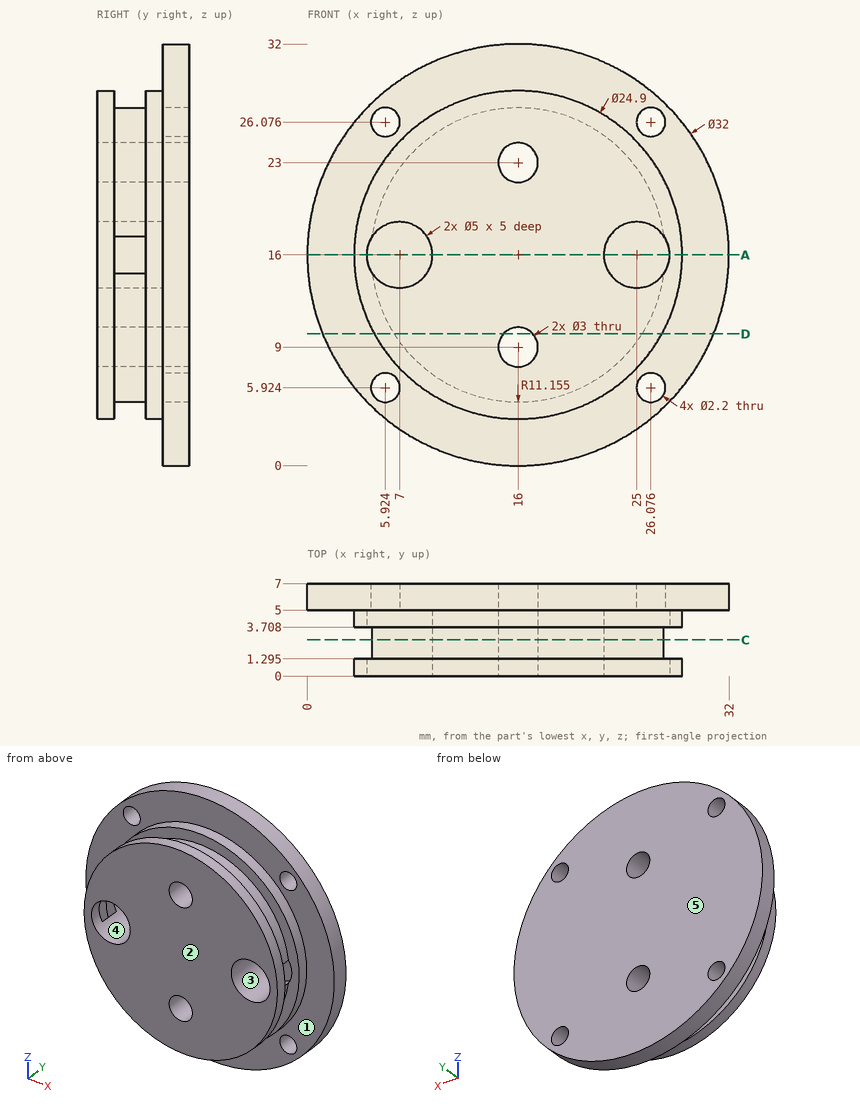
Check sheet for the drawn part. Datum: minimum x, y, z corner. Units: mm. A direction names the side the tool comes from. Give positions to 0.01 mm unless a question says otherwise; leave off trailing zeros. Order: outer loops, then holes, each group sorted by start corner. A loop starts at its lowest first (then second) coordinate and runs counter-clockwise, first axis right, second up. Notation, with made-up numbers: (47, 17) - (81, 17) arc R29 ccw to (81, 48) - close; hole circle Ø7 at (-14, -11.5). An arc over 180 degrees is marked (long way). Answer as a JSON object with one key per item and string values.
(1) Depth check by flat-ended pin: pin 1 Ø2.5 at (x, z) = (8, 17) entering from -Y; pin 2 Ø1 at (y, z) = (1, 26.5) entering from +X (1 decimal); pin 3 Ø3.5 at (x, z) = (5.92, 5.92) entering from -Y; pin 4 Ø4 at (x, y) = (13.5, 5) entering from -Z. Enter the tip coordinate at first touch or a pass-through.
Report:
{"pin 1": "y = 0", "pin 2": "x = 23.4", "pin 3": "y = 5", "pin 4": "z = 0.01"}
(2) Cross-section at A-A (z = 16). State how many separate pieces and enclosed holes the cut face has, then the cut area to 3 significant figures.
Report:
{"separate pieces": "3", "enclosed holes": "0", "area": "134 mm^2"}
(3) Cross-section at D-D (z = 10). Record the cut outline in (x, y) (1 decimal).
Report:
{"outline": "(1.2, 5) - (5.1, 5) - (5.1, 3.7) - (6.6, 3.7) - (6.6, 1.3) - (5.1, 1.3) - (5.1, 0) - (14.9, 0) - (14.9, 7) - (1.2, 7) - close; (17.1, 0) - (26.9, 0) - (26.9, 1.3) - (25.4, 1.3) - (25.4, 3.7) - (26.9, 3.7) - (26.9, 5) - (30.8, 5) - (30.8, 7) - (17.1, 7) - close"}
(4) Material ranges on line 1 (X direction, y = 0.5, z = 16); line 2 (X direction, y = 4.5, z = 14); line 3 (Z direction, x = 5.5, y = 5.5), recorded low to high.
Report:
{"line 1": "3.55 to 4.5, 9.5 to 22.5, 27.5 to 28.45", "line 2": "3.71 to 5.5, 8.5 to 23.5, 26.5 to 28.29", "line 3": "3.93 to 4.91, 6.94 to 25.06, 27.09 to 28.07"}
(5) Draft check along X on the marked faces 3, 4 and 5. Enter one of: released by +X, released by -X, zero draft, split by the parting line, or undercut.
Report:
{"face 3": "undercut", "face 4": "undercut", "face 5": "zero draft"}
(6) Tool access check on the marked faces 1 and 2. Record the directions out of +Z, -Z, +X, -X, +Y, -Y that give a thin tool (end or side, any length) a straight path to the whole face; none if there is none.
Report:
{"face 1": "-Y", "face 2": "+Z, -Z, +X, -X, -Y"}
(7) Cross-section at C-C (y = 2.75). Record the cut outline in (x, z) (1 decimal).
Report:
{"outline": "(4.9, 14.6) arc R11.2 ccw to (27.1, 14.6) arc R2.5 cw (long way) to (27.1, 17.4) arc R11.2 ccw to (4.9, 17.4) arc R2.5 cw (long way) to start; hole circle Ø3 at (16, 9); hole circle Ø3 at (16, 23)"}
